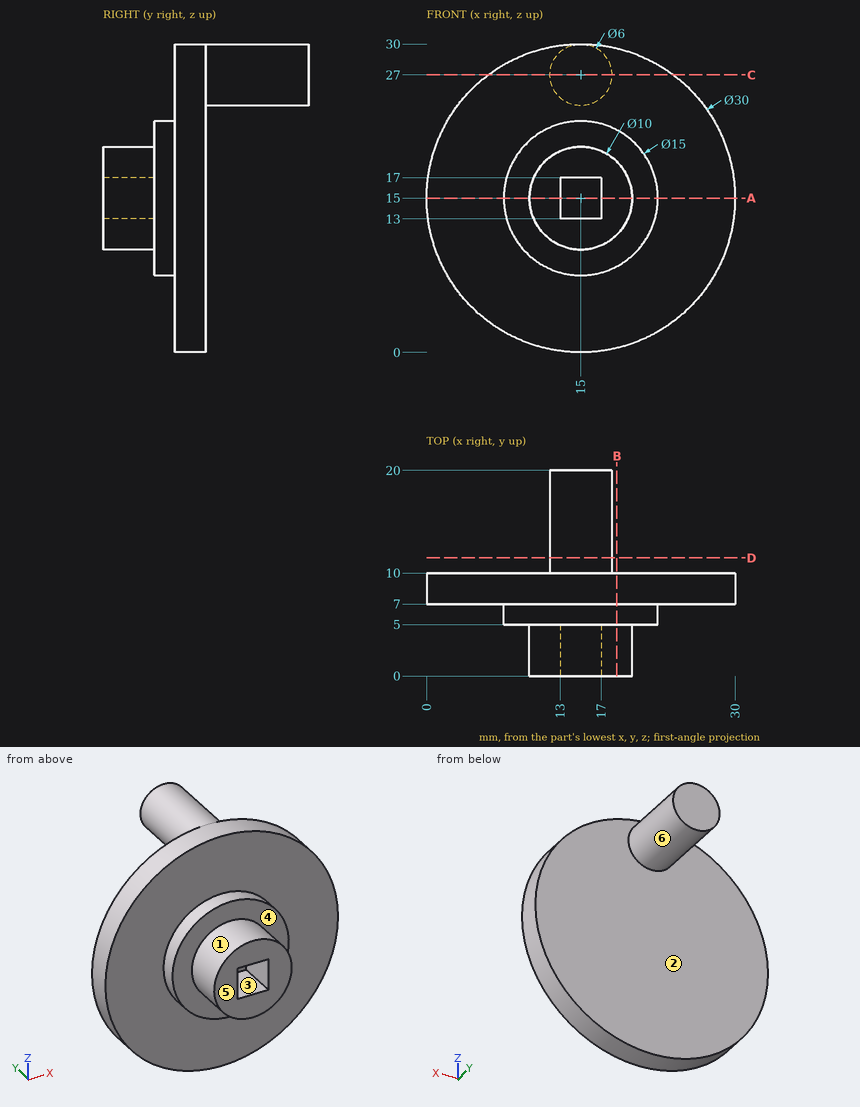
For this review, use the dimensioned drawing (mm, ordinates from the lowest corner) and the shaded views. A direction names the side the tool comes from. Round coordinates to 2 decimals unless told otherwise and drop trailing zeros. Loops run counter-clockwise (first coordinate to the right, second up) from the corner with the lowest first, then second, coordinate; pieces in that order, holes last. Notation, with made-up numbers: (23, 19.5) -> (78, 19.5) arc R15 cw to (78, 48.5) -> close; hole circle Ø8 at (70, 56.25). An arc over 180 degrees is marked (long way). Write item = value, one per line. Start each with the question number.
Item 1: Mouldability with a two-part tool opening along Z and no side actions: class the marked faces 1, 2 and 3 as released by +Z, released by -Z, zero draft, split by the parting line, or undercut.
Item 2: To check wall thickness, follow L1, parallel to Y at x = 16.5, z = 9; L2, parallel to Y at x = 19.25, z = 28.5; L3, parallel to X at y = 4.25, z = 11. State the ranges of each line that lie inside material, in increasing order.
Item 3: Take a section at A-A on z = 15. Give the boundary of the cut face in (x, y), plus the area to 3 significant figures.
Item 4: Insertion check: pin 1 (3 mm diameter, centred on y = 11, z = 24, fed in from +X); pin 2 (2 mm diameter, centred on x = 14.5, y = 3.5, fed in from -Z); pin 3 (6 mm diameter, centred on x = 10.5, y = 9.5, fed in from -Z). Each pin has a flat end and moves straight along its axis. Give the tip position at first contact, or say it passes through.
Item 5: For the marked faces 4, 5 and 6, list the 3-axis set-ups (+Z, -Z, +X, -X, +Y, -Y) from which the entire face can be reached by the end or side of a thin tool; tool diameter is ignored.
Item 6: Take a section at C-C on z = 27. Give the boundary of the cut face in (x, y).
Item 7: Take a section at B-B on x = 18.5. Give the boundary of the cut face in (y, z).
Item 8: Take a section at D-D on y = 11.5. Give the boundary of the cut face in (x, z), plus the area to 3 significant figures.
Result:
q1.face_1 = split by the parting line
q1.face_2 = zero draft
q1.face_3 = undercut
q2.L1 = 5 to 10
q2.L2 = 7 to 10
q2.L3 = 12 to 18
q3.outline = (0, 7) -> (7.5, 7) -> (7.5, 5) -> (10, 5) -> (10, 0) -> (13, 0) -> (13, 5) -> (17, 5) -> (17, 0) -> (20, 0) -> (20, 5) -> (22.5, 5) -> (22.5, 7) -> (30, 7) -> (30, 10) -> (0, 10) -> close
q3.area = 150 mm²
q4.pin_1 = 27.76
q4.pin_2 = 10
q4.pin_3 = 0.08
q5.face_4 = -Y
q5.face_5 = +Z, -Z, +X, -X, -Y
q5.face_6 = +Y
q6.outline = (6, 7) -> (24, 7) -> (24, 10) -> (18, 10) -> (18, 20) -> (12, 20) -> (12, 10) -> (6, 10) -> close
q7.outline = (0, 11.43) -> (5, 11.43) -> (5, 8.37) -> (7, 8.37) -> (7, 0.41) -> (10, 0.41) -> (10, 29.59) -> (7, 29.59) -> (7, 21.63) -> (5, 21.63) -> (5, 18.57) -> (0, 18.57) -> close
q8.outline = circle Ø6 at (15, 27)
q8.area = 28.3 mm²
